Build history of the part. All positions in model axes, mm. Face numbers are marked on the shaded views. Give positions to 0.01 mm unless a question says otherwise; leave off trailing zeros. Write each loop counter-clockwise with the first axis right and the second up, starting at its lowest first coordinate (ties: lowest second). Pieces come first, ordered by that corner, then holes.
from build123d import *

# Parameters (mm, degrees)
SKETCH1_W           = 55
SKETCH1_H           = 20
BOSS_EXTRUDE1_DEPTH = 20
M6_TAPPED_HOLE1_D   = 5
CHAMFER1_SIZE       = 1


with BuildPart() as part:
    # Sketch1 → Boss-Extrude1 (new body)
    with BuildSketch(Plane.XY):
        with Locations((-52.336320298, 28.055555556)):
            Rectangle(SKETCH1_W, SKETCH1_H)
    extrude(amount=BOSS_EXTRUDE1_DEPTH)

    # M6 Tapped Hole1 (through all)
    with Locations(Plane.XY.offset(20)):
        with Locations((-67.336320298, 28.055555556), (-37.336320298, 28.055555556)):
            Hole(M6_TAPPED_HOLE1_D / 2)

    # Chamfer1
    chamfer1_edges = [part.edges().sort_by_distance(p)[0] for p in [
        (-79.836320298, 38.055555556, 10),
        (-24.836320298, 38.055555556, 10),
        (-24.836320298, 18.055555556, 10),
        (-79.836320298, 18.055555556, 10),
    ]]
    chamfer(chamfer1_edges, length=CHAMFER1_SIZE)


solid = part.part
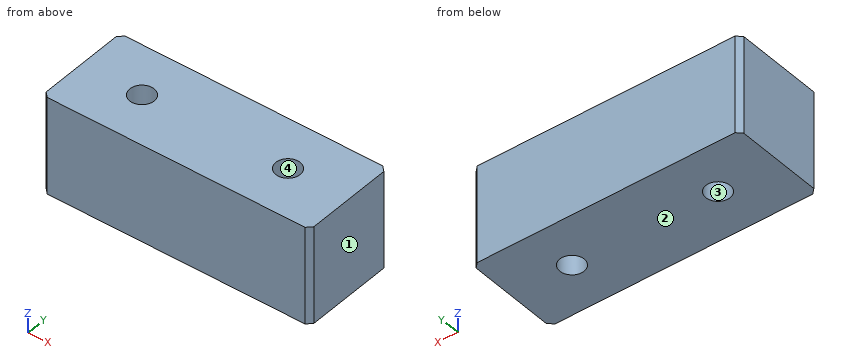
(1) Probe line 1 (Y direction, x = -37.5, z = 7.75); line 2 (X direction, y = 26.5, z = 3.5); line 3 (X direction, y = 26, z = 2). List the from-to ranges inside material, lowest first.
(2) Mould opens along X. For the marked faces 1, 2, 3 and 4 say: +X half, -X half, draft (parallel to the pull), parting line (faces both ways), or undercut.
(3) Saw through at A-A, the plane y = 29.5. List the corners of the cut face in (x, z).
(4) Saw through at B-B, the plane z = 9.75. List the corners of the cut face in (x, y).
Computed values:
1. line 1: y = 18.06 to 25.56, 30.55 to 38.06
1. line 2: x = -79.84 to -69.29, -65.38 to -39.29, -35.38 to -24.84
1. line 3: x = -79.84 to -68.76, -65.91 to -38.76, -35.91 to -24.84
2. face 1: +X half
2. face 2: draft
2. face 3: undercut
2. face 4: undercut
3. outline: (-79.84, 0) - (-69.38, 0) - (-69.38, 20) - (-79.84, 20) - close; (-65.3, 0) - (-39.38, 0) - (-39.38, 20) - (-65.3, 20) - close; (-35.3, 0) - (-24.84, 0) - (-24.84, 20) - (-35.3, 20) - close
4. outline: (-79.84, 19.06) - (-78.84, 18.06) - (-25.84, 18.06) - (-24.84, 19.06) - (-24.84, 37.06) - (-25.84, 38.06) - (-78.84, 38.06) - (-79.84, 37.06) - close; hole circle Ø5 at (-67.34, 28.06); hole circle Ø5 at (-37.34, 28.06)
